Work out the finished part from the listing and answer in its coordinate system (mm). Face numbers are marked on the shaded views. A direction names the side the tool comes from. Give positions to 0.01 mm unless a question says otherwise; leave off trailing zeros. Loops run counter-clockwise (first coordinate to the right, second up) from the corner with the lowest first, then second, coordinate; pieces in that order, holes last. Notation, with made-up numbers: (77.25, 55) - (101.25, 55) arc R26 cw to (101.25, 83) - close; hole circle Ø5 at (-36, 79). An arc over 180 degrees is marked (long way). Use CSV: the item, a comma, the result in double quotes.
from build123d import *

# Parameters (mm, degrees)
BASE_ANGLE_DEPTH             = 20
UPRIGHT_PLATE_SKETCH_W       = 40
UPRIGHT_PLATE_SKETCH_H       = 43
UPRIGHT_PLATE_DEPTH          = 7
BEARING_HUB_SKETCH_R         = 15
BEARING_HUB_SKETCH_R_2       = 11
BEARING_HUB_30_BORE_22_DEPTH = 18
GUSSET_START                 = -6
GUSSET_RIB_DEPTH             = 4


with BuildPart() as part:
    # Base Angle Profile Sketch → Base Angle (new, symmetric)
    with BuildSketch(Plane(origin=(0, 0, 0), x_dir=(0, 0, -1), z_dir=(1, 0, 0))):
        Polygon((0, 0), (32, 0), (32, 50), (25, 50), (25, 7), (0, 7), align=None)
    extrude(amount=BASE_ANGLE_DEPTH, both=True)

    # Upright Plate Sketch → Upright Plate (add)
    with BuildSketch(Plane.XY.offset(-25)):
        with Locations((0, 28.5)):
            Rectangle(UPRIGHT_PLATE_SKETCH_W, UPRIGHT_PLATE_SKETCH_H)
        with BuildLine():
            ThreePointArc((20, 50), (0, 70), (-20, 50))
            Line((-20, 50), (20, 50))
        make_face()
    extrude(amount=-UPRIGHT_PLATE_DEPTH)

    # Bearing Hub Sketch → Bearing Hub Ø30 Bore Ø22 (add)
    with BuildSketch(Plane.XY.offset(-25)):
        with Locations(Location((0, 50, 0), (0, 0, 90))):
            Circle(BEARING_HUB_SKETCH_R)
        with Locations((0, 50)):
            Circle(BEARING_HUB_SKETCH_R_2, mode=Mode.SUBTRACT)
    extrude(amount=BEARING_HUB_30_BORE_22_DEPTH)

    # Gusset Rib Sketch → Gusset Rib (add)
    with BuildSketch(Plane(origin=(20, 0, 0), x_dir=(0, 0, -1), z_dir=(1, 0, 0)).offset(GUSSET_START)):
        Polygon((5, 7), (25, 27), (25, 7), align=None)
    gusset_rib = extrude(amount=GUSSET_RIB_DEPTH)

    # Gusset Rib Mirror: Gusset Rib across plane
    add(gusset_rib.mirror(Plane(origin=(0, 0, 0), x_dir=(0, 0, 1), z_dir=(1, 0, 0))))


solid = part.part
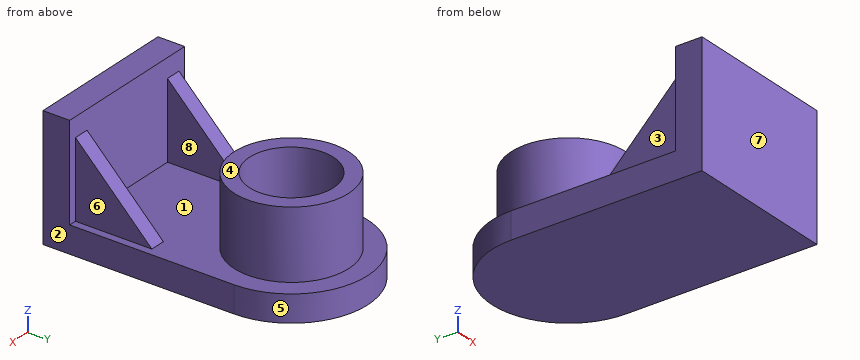
Item 1: A cutting plane is placed at C-C on y = 21.5. Determine the outline of the cut face in (x, z).
Determined:
outline,"(-20, -32) - (20, -32) - (20, -25) - (18, -25) - (18, -19.5) - (14, -19.5) - (14, -25) - (-14, -25) - (-14, -19.5) - (-18, -19.5) - (-18, -25) - (-20, -25) - close"
Item 2: Given P1, Ø1.5, axis at y = 60.5, z = -7, coming from the +X side; P2, Ø10, axis at y = 18, z = -19.5, coming from the +X side; P3, Ø3, axis at x = -9.5, z = -15, coming from the +Y side, each flat-ended and moving along its own axis, determine where each tip first touches the part or whether it passes through.
Determined:
P1,"stops at x = 11.4"
P2,"stops at x = 18"
P3,"stops at y = 62.69"
Item 3: Find the intervals of material crossed by line 1 (X direction, y = 13.5, z = -13); line 2 (Y direction, x = 3, z = -2); line 3 (Z direction, x = 7, y = 42), in increasing order.
Determined:
line 1,"x = -18 to -14, 14 to 18"
line 2,"y = 0 to 7"
line 3,"z = -32 to -25"
Item 4: The mould has two halves that part along Y. Classify the marked faces 5, 6, 7 and 8: pulls with the +Y half, pulls with the -Y half, needs draft (parallel to the pull), parting line crosses it, or undercut.
Determined:
face 5,"pulls with the +Y half"
face 6,"needs draft"
face 7,"pulls with the -Y half"
face 8,"undercut"
Item 5: A cutting plane is placed at A-A on z = -8. Determine the outline of the cut face in (x, y).
Determined:
outline,"(-20, 0) - (20, 0) - (20, 7) - (18, 7) - (18, 10) - (14, 10) - (14, 7) - (-14, 7) - (-14, 10) - (-18, 10) - (-18, 7) - (-20, 7) - close; circle Ø30 at (0, 50); hole circle Ø22 at (0, 50)"
Item 6: A cutting plane is placed at D-D on z = -22. Determine the outline of the cut face in (x, y), and give its area (3 significant figures).
Determined:
outline,"(-20, 0) - (20, 0) - (20, 7) - (18, 7) - (18, 24) - (14, 24) - (14, 7) - (-14, 7) - (-14, 24) - (-18, 24) - (-18, 7) - (-20, 7) - close; circle Ø30 at (0, 50); hole circle Ø22 at (0, 50)"
area,"743 mm²"
Item 7: For the marked faces 1, 2, 3 and 4, determine the directions among +Z, -Z, +X, -X, +Y, -Y from which every point of the face is accessible in a straight line to the end or side of a thin tool.
Determined:
face 1,"+Z"
face 2,"+Z, -Z, +X, +Y, -Y"
face 3,"+Z, -X, +Y"
face 4,"+Z, +X, -X, +Y"
Item 8: A cutting plane is placed at B-B on x = 0. Determine the outline of the cut face in (y, z).
Determined:
outline,"(0, -32) - (70, -32) - (70, -25) - (65, -25) - (65, -7) - (61, -7) - (61, -25) - (39, -25) - (39, -7) - (35, -7) - (35, -25) - (7, -25) - (7, 0) - (0, 0) - close"
